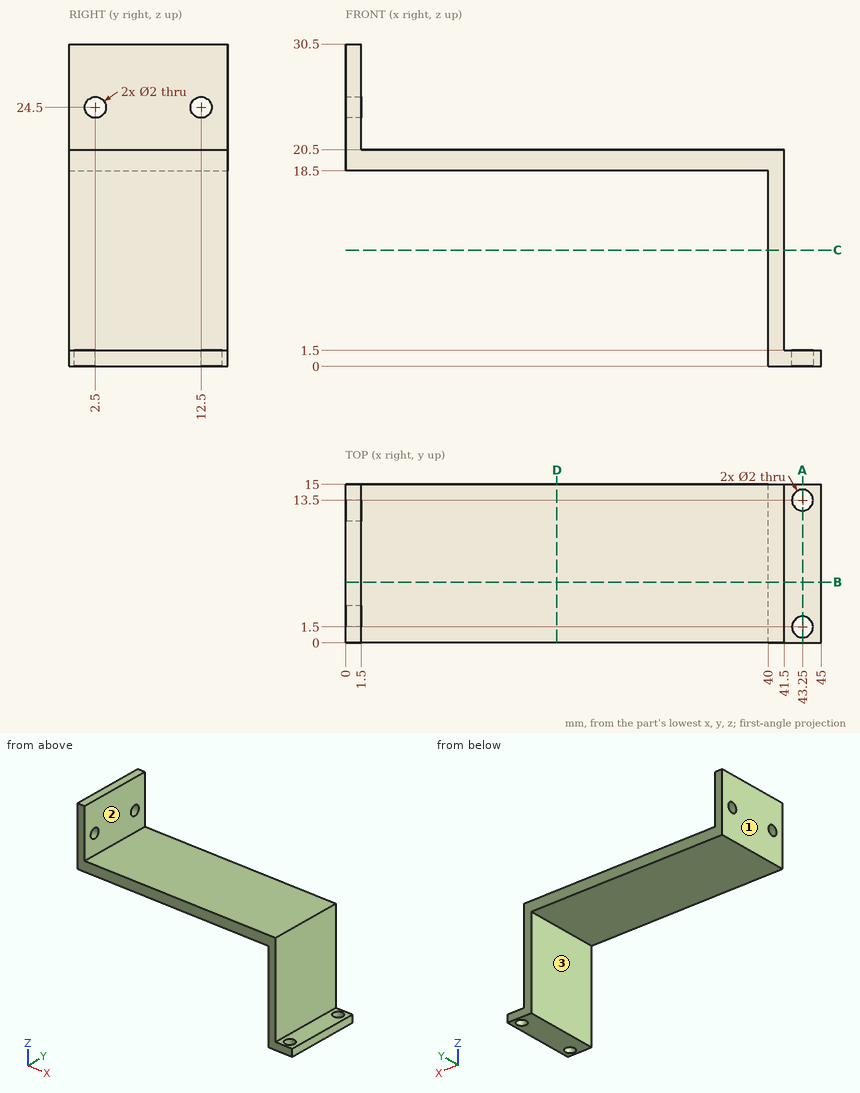
The figure shows three views and two pictorial views of one solid part (mm, origin at its lowest corner). Answer the questions. A direction names the side the tool comes from. Coordinates: 2 decimals unless noted, no trailing zeros. Write each loop counter-clockwise with the first axis right and the second up, starting at its lowest first coordinate (ties: lowest second). Pieces come first, ordered by that corner, then holes. Notation, with made-up numbers: (60, 16.5) -> (93, 16.5) arc R8 ccw to (93, 21.5) -> close; hole circle Ø1 at (13.25, 86.5). An arc over 180 degrees is marked (long way). Answer as a JSON object with one key per item and string values.
Q1. Consider line 1 (Y direction, x = 0.5, z = 24.5); line 2 (Y direction, x = 1, z = 24); line 3 (Z direction, x = 11, y = 2.75). Determine where each line is inside the solid, lowest interval first. Write a range as [from, to].
The answers:
{"line 1": "y = [0, 1.5], [3.5, 11.5], [13.5, 15]", "line 2": "y = [0, 1.63], [3.37, 11.63], [13.37, 15]", "line 3": "z = [18.5, 20.5]"}
Q2. The part is cut by section B-B on y = 5.75. Give the vertices of the cut face in (x, z), then the cut area to 3 significant figures.
The answers:
{"outline": "(0, 18.5) -> (40, 18.5) -> (40, 0) -> (45, 0) -> (45, 1.5) -> (41.5, 1.5) -> (41.5, 20.5) -> (1.5, 20.5) -> (1.5, 30.5) -> (0, 30.5) -> close", "area": "131 mm2"}
Q3. Flat-ended cylindrical pins translate along their axes: pin 1 Ø6 at (y, z) = (7.5, 11) entering from -X; pin 2 Ø4.5 at (x, y) = (23.5, 11) entering from -Z; pin 3 Ø3 at (x, y) = (43.25, 1.5) entering from +Z; pin 4 Ø1.8 at (x, y) = (43.25, 13.5) entering from -Z. Find the tip coordinate at first contact, or state that the pin passes through.
The answers:
{"pin 1": "stops at x = 40", "pin 2": "stops at z = 18.5", "pin 3": "stops at z = 1.5", "pin 4": "passes through"}
Q4. A tool of negligible diameter and unlimited length cuts with its end or side. For the marked faces 1, 2 and 3, from which of +Z, -Z, +X, -X, +Y, -Y can it reach the whole face along a straight path? Write none if from no direction.
The answers:
{"face 1": "+Z, -Z, -X, +Y, -Y", "face 2": "+Z, +X, +Y, -Y", "face 3": "-Z, -X, +Y, -Y"}
Q5. The part is cut by section D-D on x = 20. Give the vertices of the cut face in (y, z), then the cut area to 3 significant figures.
The answers:
{"outline": "(0, 18.5) -> (15, 18.5) -> (15, 20.5) -> (0, 20.5) -> close", "area": "30.0 mm2"}
Q6. The part is cut by section A-A on x = 43.25. Give the vertices of the cut face in (y, z), then the cut area to 3 significant figures.
The answers:
{"outline": "(0, 0) -> (0.5, 0) -> (0.5, 1.5) -> (0, 1.5) -> close; (2.5, 0) -> (12.5, 0) -> (12.5, 1.5) -> (2.5, 1.5) -> close; (14.5, 0) -> (15, 0) -> (15, 1.5) -> (14.5, 1.5) -> close", "area": "16.5 mm2"}
Q7. The part is cut by section C-C on z = 11. Give the vertices of the cut face in (x, y).
The answers:
{"outline": "(40, 0) -> (41.5, 0) -> (41.5, 15) -> (40, 15) -> close"}
